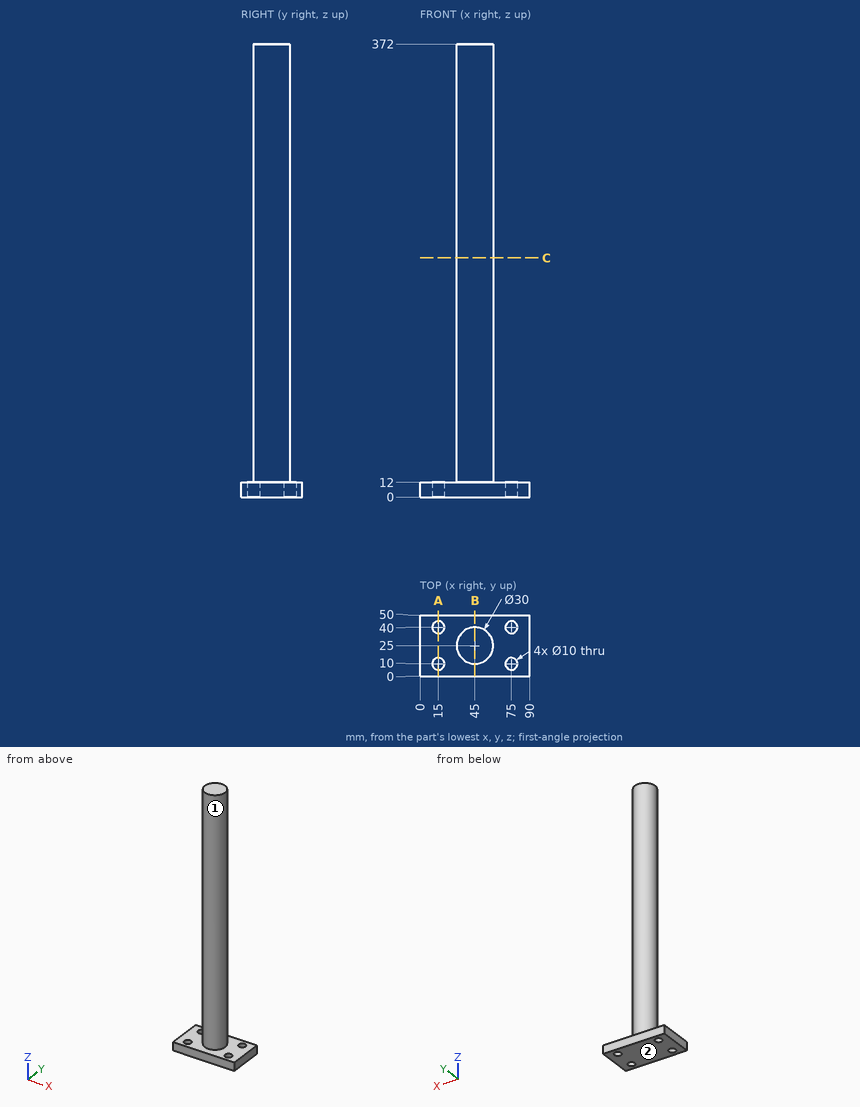
Could you check a few things on this drawing? It's one solid part, dimensions in mm from its lowest x, y, z. A direction names the side the tool comes from. Coordinates: 2 decimals unless noted, no trailing zeros. Order: outer loops, then holes, each group sorted by start corner. A loop starts at its lowest first (then second) coordinate and runs counter-clockwise, first axis right, second up.
1. If we section it at A-A (x = 15): Please give me the cut outline in (y, z), then the cut area to 3 significant figures.
2. For the marked faces 1 and 2, which set-ups out of +Z, -Z, +X, -X, +Y, -Y let a thin tool reach every point of the face, with its end or its side?
3. I'm going to push flat-ended pins straight in: pin 1 (12 mm diameter, centred on y = 27, z = 50, fed in from +X); pin 2 (6 mm diameter, centred on x = 45, y = 6.5, fed in from +Z); pin 3 (8 mm diameter, centred on x = 42, z = 96, fed in from +Y). Where does each tip first touch, or does it pass through?
4. I need wall thicknesses on line 1 (Y direction, x = 15, z = 6); line 2 (Z direction, x = 85, y = 33); line 3 (Y direction, x = 57, z = 156). Which ranges of each line are inside material? Lowest first, please.
5. If we section it at B-B (x = 45): Please give me the cut outline in (y, z).
6. If we section it at C-C (z = 196.5): Please give me the cut outline in (x, y), then the cut area to 3 significant figures.
Entries:
1. outline: (0, 0) - (5, 0) - (5, 12) - (0, 12) - close; (15, 0) - (35, 0) - (35, 12) - (15, 12) - close; (45, 0) - (50, 0) - (50, 12) - (45, 12) - close
1. area: 360 mm2
2. face 1: +Z
2. face 2: -Z, +X, -X, +Y, -Y
3. pin 1: stops at x = 60
3. pin 2: stops at z = 12
3. pin 3: stops at y = 40
4. line 1: y = 0 to 5, 15 to 35, 45 to 50
4. line 2: z = 0 to 12
4. line 3: y = 16 to 34
5. outline: (0, 0) - (50, 0) - (50, 12) - (40, 12) - (40, 372) - (10, 372) - (10, 12) - (0, 12) - close
6. outline: circle Ø30 at (45, 25)
6. area: 707 mm2
